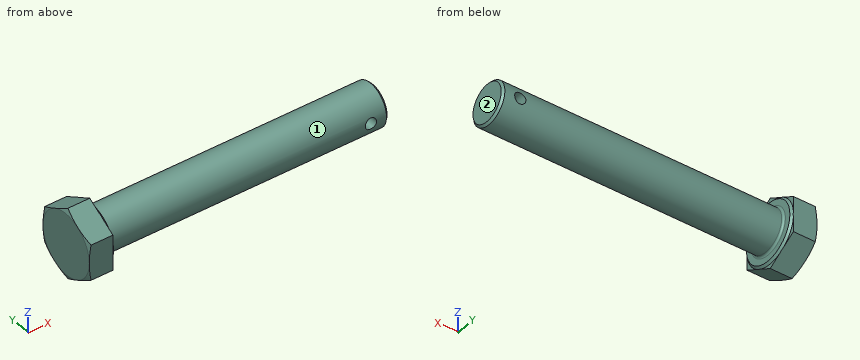
```python
from build123d import *

# Parameters (mm, degrees)
BASEHEAD_DEPTH  = 7.32
SKETCH5_R       = 6
BASEBODY_DEPTH  = 80
CHAMFER1_SIZE   = 0.6
HOLE_DEPTH      = 89.363764774
HOLE_DEPTH_BACK = 89.363764774
SKETCH6_R       = 1.6
HEADFILLET_R    = 0.6


with BuildPart() as part:
    # Sketch2 → BaseHead (new body)
    with BuildSketch(Plane(origin=(0, 0, 0), x_dir=(0, 0, -1), z_dir=(1, 0, 0))):
        Polygon((10.236420273, 0), (5.118210136, 8.865), (-5.118210136, 8.865), (-10.236420273, 0), (-5.118210136, -8.865), (5.118210136, -8.865), align=None)
    extrude(amount=BASEHEAD_DEPTH)

    # Sketch3 → BearingFace (revolve, cut)
    with BuildSketch(Plane(origin=(0, 0, 0), x_dir=(1, 0, 0), z_dir=(0, 1, 0)), mode=Mode.PRIVATE) as bearingface_sk:
        Polygon((7.32, 10.236420273), (7.32, 8.315), (6.72, 8.915), (6.72, 10.236420273), align=None)
    revolve(bearingface_sk.sketch.rotate(Axis((-0.957090588, 0, 0), (1, 0, 0)), 180), axis=Axis((-0.957090588, 0, 0), (1, 0, 0)), mode=Mode.SUBTRACT)

    # Sketch4 → HeadChamfer (revolve, cut)
    with BuildSketch(Plane(origin=(0, 0, 0), x_dir=(1, 0, 0), z_dir=(0, 1, 0))):
        Polygon((0, 10.236420273), (0.499156158, 10.236420273), (0, 8.865), align=None)
    revolve(axis=Axis((-0.493528746, 0, 0), (1, 0, 0)), mode=Mode.SUBTRACT)

    # Sketch5 → BaseBody (add)
    with BuildSketch(Plane(origin=(7.32, 0, 0), x_dir=(0, 0, -1), z_dir=(1, 0, 0))):
        Circle(SKETCH5_R)
    extrude(amount=BASEBODY_DEPTH)

    # Chamfer1
    chamfer1_edges = [part.edges().sort_by_distance(p)[0] for p in [
        (87.32, 0, 6),
    ]]
    chamfer(chamfer1_edges, length=CHAMFER1_SIZE)

    # Sketch6 → Hole (cut, two sides: drawn at the far end of the back side and taken through both)
    with BuildSketch(Plane(origin=(0, 0, 0), x_dir=(1, 0, 0), z_dir=(0, 1, 0)).offset(-HOLE_DEPTH_BACK)):
        with Locations(Location((82.32, 0, 0), (0, 0, 270))):
            Circle(SKETCH6_R)
    extrude(amount=HOLE_DEPTH + HOLE_DEPTH_BACK, mode=Mode.SUBTRACT)

    # HeadFillet
    headfillet_edges = [part.edges().sort_by_distance(p)[0] for p in [
        (7.32, 0, 6),
    ]]
    fillet(headfillet_edges, radius=HEADFILLET_R)


solid = part.part
```
Source: CAD feature listing. Evaluate the final solid. Frame: model axes, mm. Face numbers are marked on the shaded views. A direction names the side the tool comes from. Give positions to 0.01 mm unless a question says otherwise; leave off trailing zeros. Loops run counter-clockwise (first coordinate to the right, second up) from the corner with the lowest first, then second, coordinate; pieces in that order, holes last. Notation, with made-up numbers: (-5.75, 38.5) -> (6.25, 38.5) arc R22 ccw to (6.25, 66.5) -> close; hole circle Ø4 at (-23, 9.25). An arc over 180 degrees is marked (long way). Use a Markdown table: item, result. Add a question column.
(1) Section query A-A (x = 52.5). Output: boundary loops of the cut face in (y, z).
(2) Section query B-B (x = 82.32). Output: boundary loops of the cut face in (y, z), then the cut area to 3 significant figures.
(3) Access query for the marked faces 1 and 2. Directions: +Z, -Z, +X, -X, +Y, -Y. A direction counts if a zero-diameter tool reaches every point of the face in a straight line with its end or side. Return the directions, or none.
(4) Ray query, line 1 (X direction, y = -1, z = 0); line 2 (Z direction, x = 82.32, y = -1); line 3 (Z direction, x = 82.32, y = 2). Return the intervals inside material, ascending.
(5) First-contact query: pin 1 Ø1.9 at (x, z) = (82.32, 0) entering from -Y; pin 2 Ø0.6 at (y, z) = (0, 9.5) entering from +X; pin 3 Ø4 at (x, z) = (14, -2) entering from -Y; pin 4 Ø3 at (x, y) = (44, 4) entering from -Z. Flat tips, straight axial feed; report the tip coordinate or a pass-through.
Checked values:
| question | item | result |
|---|---|---|
| 1 | outline | circle Ø12 at (0, 0) |
| 2 | outline | (-5.78, -1.6) arc R6 ccw to (5.78, -1.6) -> close; (-5.78, 1.6) -> (5.78, 1.6) arc R6 ccw to start |
| 2 | area | 75.2 mm^2 |
| 3 | face 1 | +X |
| 3 | face 2 | +Z, -Z, +X, +Y, -Y |
| 4 | line 1 | 0 to 80.72, 83.92 to 87.32 |
| 4 | line 2 | -5.92 to -1.6, 1.6 to 5.92 |
| 4 | line 3 | -5.66 to -1.6, 1.6 to 5.66 |
| 5 | pin 1 | through |
| 5 | pin 2 | x = 6.72 |
| 5 | pin 3 | y = -6 |
| 5 | pin 4 | z = -5.45 |
